Geometry check sheet. Reference: drawing and pictorial views, mm from the part's lowest x, y, z. A direction names the side the tool comes from. Round coordinates to 2 decimals unless told otherwise and drop trailing zeros. Write each loop counter-clockwise with the first axis right and the second up, starting at its lowest first coordinate (ties: lowest second). Pieces come first, ordered by that corner, then holes. Notation, with made-up numbers: M 39.5,51 L 63.5,51 A35 ccw 63.5,83 Z; hole C 12.5,-21.75 d8. An arc over 180 degrees is marked long. One line per question, with ' | ' between items.
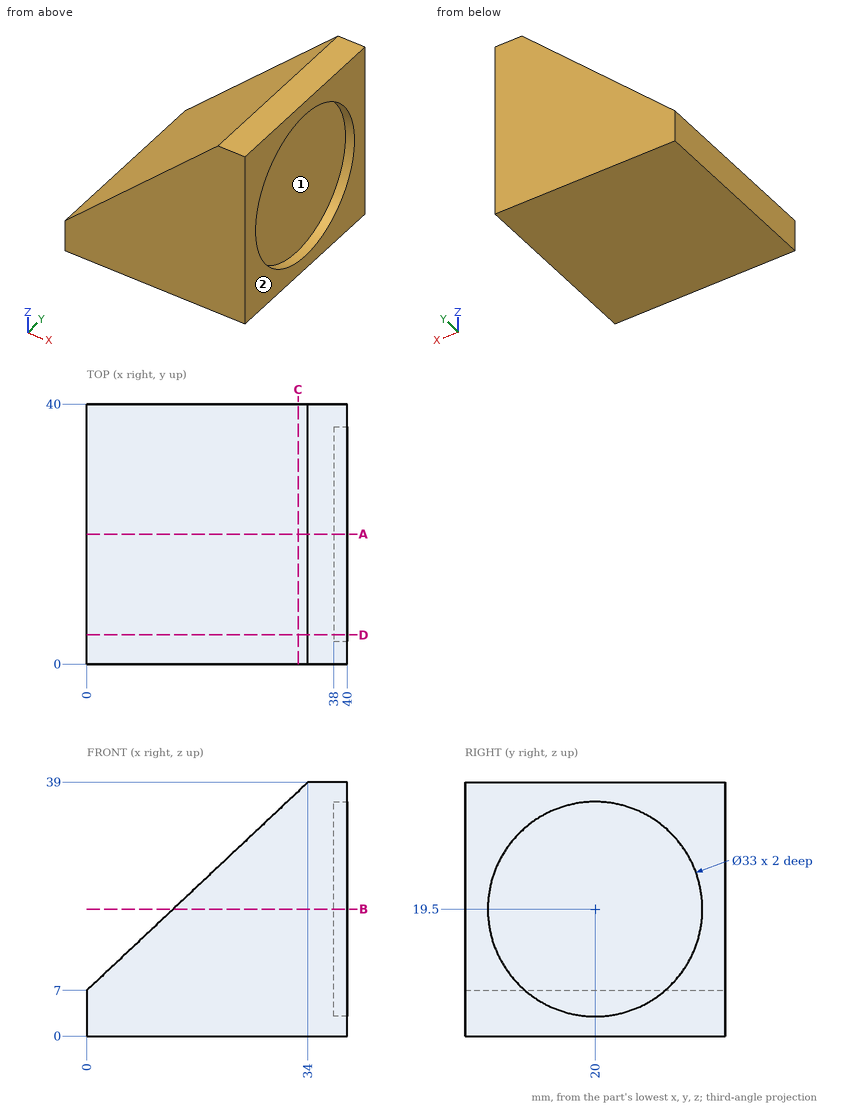
1. Section check D-D, the plane y = 4.5. Record the cut outline in (x, z), then the cut area to 3 significant figures.
Results:
outline: M 0,0 L 40,0 L 40,13.84 L 38,13.84 L 38,25.16 L 40,25.16 L 40,39 L 34,39 L 0,7 Z | area: 993 mm2
2. Section check C-C, the plane x = 32.5. Record the cut outline in (y, z), then the cut area to 3 significant figures.
Results:
outline: M 0,0 L 40,0 L 40,37.59 L 0,37.59 Z | area: 1,500 mm2
3. Thickness scan on line 1 (Y direction, x = 39.25, z = 19.5); line 2 (Z direction, x = 27.5, y = 3); line 3 (X direction, y = 29.5, z = 35). Record the ranges inside material, lowest first.
Results:
line 1: y = 0 to 3.5, 36.5 to 40 | line 2: z = 0 to 32.88 | line 3: x = 29.75 to 40
4. Section check A-A, the plane y = 20. Record the cut outline in (x, z), then the cut area to 3 significant figures.
Results:
outline: M 0,0 L 40,0 L 40,3 L 38,3 L 38,36 L 40,36 L 40,39 L 34,39 L 0,7 Z | area: 950 mm2
5. Go/stop test with flat-tipped pins: P1, Ø6, axis at x = 24, y = 19, coming from the +Z side; P2, Ø1, axis at x = 4.5, y = 5.5, coming from the +Z side; P3, Ø10, axis at y = 17, z = 15.5, coming from the +X side. Record where each tip stops, or that it passes through.
Results:
P1: stops at z = 32.41 | P2: stops at z = 11.71 | P3: stops at x = 38
6. Tool access check on the marked faces 1 and 2. Record the directions out of +Z, -Z, +X, -X, +Y, -Y that give a thin tool (end or side, any length) a straight path to the whole face; none if there is none.
Results:
face 1: +X | face 2: +Z, -Z, +X, +Y, -Y
7. Section check B-B, the plane z = 19.5. Record the cut outline in (x, y), then the cut area to 3 significant figures.
Results:
outline: M 13.28,0 L 40,0 L 40,3.5 L 38,3.5 L 38,36.5 L 40,36.5 L 40,40 L 13.28,40 Z | area: 1,000 mm2
